Design review of the part shown in the three views and the two pictorial views. Dimensions are in mm from the part's minimum x, y and z. A direction names the side the tool comes from. Coordinates: 2 decimals unless noted, no trailing zeros. Write each loop counter-clockwise with the first axis right and the second up, starting at its lowest first coordinate (ties: lowest second). Pieces come first, ordered by that corner, then holes. Notation, with made-up numbers: (-15, 49) -> (39, 49) arc R28 cw to (39, 83) -> close; hole circle Ø4 at (41, -22). An arc over 180 degrees is marked (long way). Write item = value, one per line. Start each with the question number.
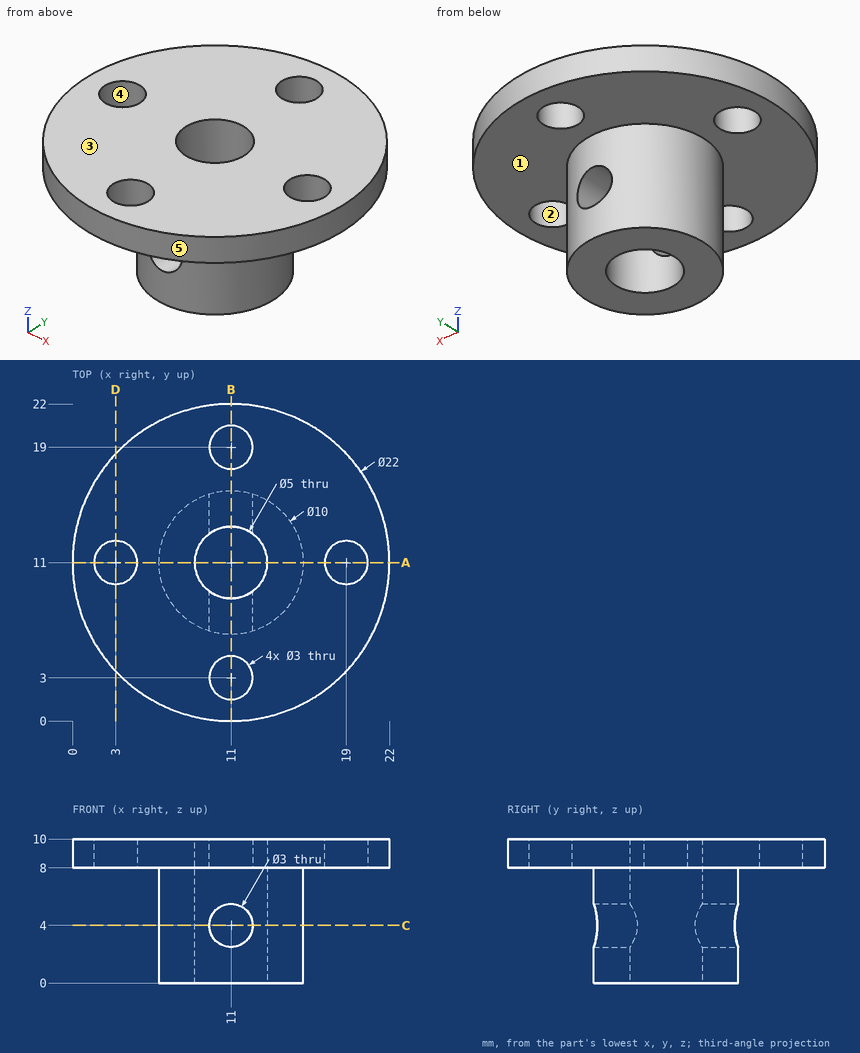
(1) Take a section at C-C, the plane z = 4. State the section outline as (x, y) points.
(2) For the marked faces 1 and 2, list the 3-axis set-ups (+Z, -Z, +X, -X, +Y, -Y) from which the entire face can be reached by the end or side of a thin tool; tool diameter is ignored.
(3) For pin 1 Ø5 at (x, z) = (11.5, 8) entering from +Y; pin 2 Ø4 at (x, z) = (11, 4) entering from +Y; pin 3 Ø6 at (x, z) = (12, 1) entering from -Y; pin 4 Ø4 at (x, z) = (14.5, 7) entering from -Y, all flat-tipped, find the tip position at first contact; note any pin that passes through.
(4) Take a section at A-A, the plane y = 11. State the section outline as (x, z) points.
(5) For line 1 (Y direction, x = 11, z = 8.9); line 2 (Z direction, x = 11, y = 13.85); line 3 (Z direction, x = 9.25, y = 17), list the stretches that pass through material, from the lowest coordinate up.
(6) Take a section at B-B, the plane x = 11. State the section outline as (y, z) points, then the cut area to 3 significant figures.
(7) Take a section at D-D, the plane x = 3. State the section outline as (y, z) points.
(8) Mouldability with a two-part tool opening along Y and no side actions: class the marked faces 3, 4 and 5 as pulls with the +Y half, pulls with the -Y half, needs draft (parallel to the pull), parting line crosses it, or undercut.
Report:
q1.outline = (9.5, 6.23) -> (9.5, 9) arc R2.5 cw to (9.5, 13) -> (9.5, 15.77) arc R5 ccw to start; (12.5, 6.23) arc R5 ccw to (12.5, 15.77) -> (12.5, 13) arc R2.5 cw to (12.5, 9) -> close
q2.face_1 = -Z
q2.face_2 = +Z, -Z
q3.pin_1 = 22
q3.pin_2 = 16
q3.pin_3 = 6
q3.pin_4 = 0.14
q4.outline = (0, 8) -> (1.5, 8) -> (1.5, 10) -> (0, 10) -> close; (4.5, 8) -> (6, 8) -> (6, 0) -> (8.5, 0) -> (8.5, 10) -> (4.5, 10) -> close; (13.5, 0) -> (16, 0) -> (16, 8) -> (17.5, 8) -> (17.5, 10) -> (13.5, 10) -> close; (20.5, 8) -> (22, 8) -> (22, 10) -> (20.5, 10) -> close
q5.line_1 = 0 to 1.5, 4.5 to 8.5, 13.5 to 17.5, 20.5 to 22
q5.line_2 = 0 to 2.5, 5.5 to 10
q5.line_3 = 8 to 10
q6.outline = (0, 8) -> (1.5, 8) -> (1.5, 10) -> (0, 10) -> close; (4.5, 8) -> (6, 8) -> (6, 5.5) -> (8.5, 5.5) -> (8.5, 10) -> (4.5, 10) -> close; (6, 0) -> (8.5, 0) -> (8.5, 2.5) -> (6, 2.5) -> close; (13.5, 0) -> (16, 0) -> (16, 2.5) -> (13.5, 2.5) -> close; (13.5, 5.5) -> (16, 5.5) -> (16, 8) -> (17.5, 8) -> (17.5, 10) -> (13.5, 10) -> close; (20.5, 8) -> (22, 8) -> (22, 10) -> (20.5, 10) -> close
q6.area = 47.0 mm2
q7.outline = (3.45, 8) -> (9.5, 8) -> (9.5, 10) -> (3.45, 10) -> close; (12.5, 8) -> (18.55, 8) -> (18.55, 10) -> (12.5, 10) -> close
q8.face_3 = needs draft
q8.face_4 = undercut
q8.face_5 = parting line crosses it
